from build123d import *

# Parameters (mm, degrees)
BOSS_EXTRUDE1_DEPTH            = 15
BOSS_EXTRUDE2_DEPTH            = 310
F_14_0_14_DIAMETER_HOLE1_D     = 14
F_14_0_14_DIAMETER_HOLE1_DEPTH = 15


with BuildPart() as part:
    # Sketch1 → Boss-Extrude1 (new body)
    with BuildSketch(Plane(origin=(0, 0, 0), x_dir=(0, 0, -1), z_dir=(1, 0, 0))):
        Polygon((0, 150), (10, 160), (150, 160), (160, 150), (160, 10), (150, 0), (10, 0), (0, 10), align=None)
    boss_extrude1 = extrude(amount=BOSS_EXTRUDE1_DEPTH)

    # Sketch2 → Boss-Extrude2 (add)
    with BuildSketch(Plane(origin=(15, 0, 0), x_dir=(0, 0, -1), z_dir=(1, 0, 0))):
        with BuildLine():
            Line((46, 130), (114, 130))
            ThreePointArc((114, 130), (125.313708499, 125.313708499), (130, 114))
            Line((130, 114), (130, 46))
            ThreePointArc((130, 46), (125.313708499, 34.686291501), (114, 30))
            Line((114, 30), (46, 30))
            ThreePointArc((46, 30), (34.686291501, 34.686291501), (30, 46))
            Line((30, 46), (30, 114))
            ThreePointArc((30, 114), (34.686291501, 125.313708499), (46, 130))
        make_face()
        with BuildLine():
            Line((46, 122), (114, 122))
            ThreePointArc((114, 122), (119.656854249, 119.656854249), (122, 114))
            Line((122, 114), (122, 46))
            ThreePointArc((122, 46), (119.656854249, 40.343145751), (114, 38))
            Line((114, 38), (46, 38))
            ThreePointArc((46, 38), (40.343145751, 40.343145751), (38, 46))
            Line((38, 46), (38, 114))
            ThreePointArc((38, 114), (40.343145751, 119.656854249), (46, 122))
        make_face(mode=Mode.SUBTRACT)
    extrude(amount=BOSS_EXTRUDE2_DEPTH)

    # Mirror1: Boss-Extrude1 across plane
    add(boss_extrude1.mirror(Plane(origin=(170, 0, 0), x_dir=(0, 0, 1), z_dir=(1, 0, 0))))

    # Ø14.0 (14) Diameter Hole1
    with Locations(Plane(origin=(15, 140, -140), x_dir=(0, 0, 1), z_dir=(1, 0, 0))):
        with Locations((0, 0), (0, 120), (120, 0), (120, 120)):
            Hole(F_14_0_14_DIAMETER_HOLE1_D / 2, depth=F_14_0_14_DIAMETER_HOLE1_DEPTH)


solid = part.part
The model under review builds one solid part; all positions refer to its coordinate system, in mm. A direction names the side the tool comes from. Round coordinates to 2 decimals unless told otherwise and drop trailing zeros. Write each loop counter-clockwise with the first axis right and the second up, starting at its lowest first coordinate (ties: lowest second). Pieces come first, ordered by that corner, then holes. Notation, with made-up numbers: (59, -10) -> (93, -10) arc R35 cw to (93, 22) -> close; hole circle Ø11 at (46, 9). An arc over 180 degrees is marked (long way). Answer as a JSON object with one key per item and string values.
1. We need section C-C on z = -90. State the section outline as (x, y) points.
Results found:
{"outline": "(0, 0) -> (15, 0) -> (15, 30) -> (325, 30) -> (325, 0) -> (340, 0) -> (340, 160) -> (325, 160) -> (325, 130) -> (15, 130) -> (15, 160) -> (0, 160) -> close; hole (15, 38) -> (325, 38) -> (325, 122) -> (15, 122) -> close"}
2. We need section B-B on y = 20. State the section outline as (x, z) points.
Results found:
{"outline": "(0, -160) -> (15, -160) -> (15, -147) -> (0, -147) -> close; (0, -133) -> (15, -133) -> (15, -27) -> (0, -27) -> close; (0, -13) -> (15, -13) -> (15, 0) -> (0, 0) -> close; (325, -160) -> (340, -160) -> (340, 0) -> (325, 0) -> close"}
3. We need section A-A on z = -140. State the section outline as (x, y) points.
Results found:
{"outline": "(0, 0) -> (15, 0) -> (15, 13) -> (0, 13) -> close; (0, 27) -> (15, 27) -> (15, 133) -> (0, 133) -> close; (0, 147) -> (15, 147) -> (15, 160) -> (0, 160) -> close; (325, 0) -> (340, 0) -> (340, 160) -> (325, 160) -> close"}
4. Clearance check with flat-ended pins moving along their axes: pin 1 (20.5 mm diameter, centred on x = 206, z = -63.5, fed in from -Y); pin 2 (2 mm diameter, centred on x = 170, y = 79.5, fed in from -Z); pin 3 (8.5 mm diameter, centred on y = 20, z = -20, fed in from -X). State where each tip first meets the part, or that it passes through.
Results found:
{"pin 1": "stops at y = 30", "pin 2": "stops at z = -130", "pin 3": "stops at x = 325"}
5. To check wall thickness, follow line 1 along Y through (x, z) = (4.25, -140); line 2 along Z through (x, y) = (5, 140); line 3 along Y through (x, z) = (197, -101). State the ranges of each line that lie inside material, in increasing order.
Results found:
{"line 1": "y = 0 to 13, 27 to 133, 147 to 160", "line 2": "z = -160 to -147, -133 to -27, -13 to 0", "line 3": "y = 30 to 38, 122 to 130"}
6. The part is to be moulded in two halves that separate along Y. For faces 1 (the face through (168, 122, -80)), 2 (the face through (340, 81, -81)), 3 (the face through (7, 0, -81)), say which applies: pulls with the +Y half, pulls with the -Y half, needs draft (parallel to the pull), parting line crosses it, or undercut.
Results found:
{"face 1": "undercut", "face 2": "needs draft", "face 3": "pulls with the -Y half"}
7. We need section D-D on x = 126. State the section outline as (y, z) points.
Results found:
{"outline": "(30, -114) arc R16 ccw to (46, -130) -> (114, -130) arc R16 ccw to (130, -114) -> (130, -46) arc R16 ccw to (114, -30) -> (46, -30) arc R16 ccw to (30, -46) -> close; hole (38, -114) arc R8 ccw to (46, -122) -> (114, -122) arc R8 ccw to (122, -114) -> (122, -46) arc R8 ccw to (114, -38) -> (46, -38) arc R8 ccw to (38, -46) -> close"}
8. Machinability: for faces 4 (the face through (168, 130, -80)), 5 (the face through (333, 160, -79)), 6 (the face through (167.83, 34.563, -34.811)), 7 (the face through (167.83, 119.594, -40.281)), 8 (the face through (7, 140, -13)), which of the approach directions +Z, -Z, +X, -X, +Y, -Y give a long, thin tool a straight path to every point of the face, cutting with its end or side? Answer none if there is none.
Results found:
{"face 4": "+Z, -Z, +Y", "face 5": "+Z, -Z, +X, -X, +Y", "face 6": "+Z, -Y", "face 7": "none", "face 8": "-X"}
